The drawing under review shows one solid part. Ordinate dimensions are in mm from its lowest x, y, z. Round coordinates to 2 decimals unless told otherwise and drop trailing zeros. Order: outer loops, then holes, each group sorted by start corner. A loop starts at its lowest first (then second) coordinate and runs counter-clockwise, first axis right, second up. Notation, with made-up numbers: (84.5, 82) -> (118.5, 82) arc R29 cw to (118.5, 116) -> close; hole circle Ø5 at (33, -5). An arc over 180 degrees is marked (long way). Put each result on its own line as item: value. Start each with the question number.
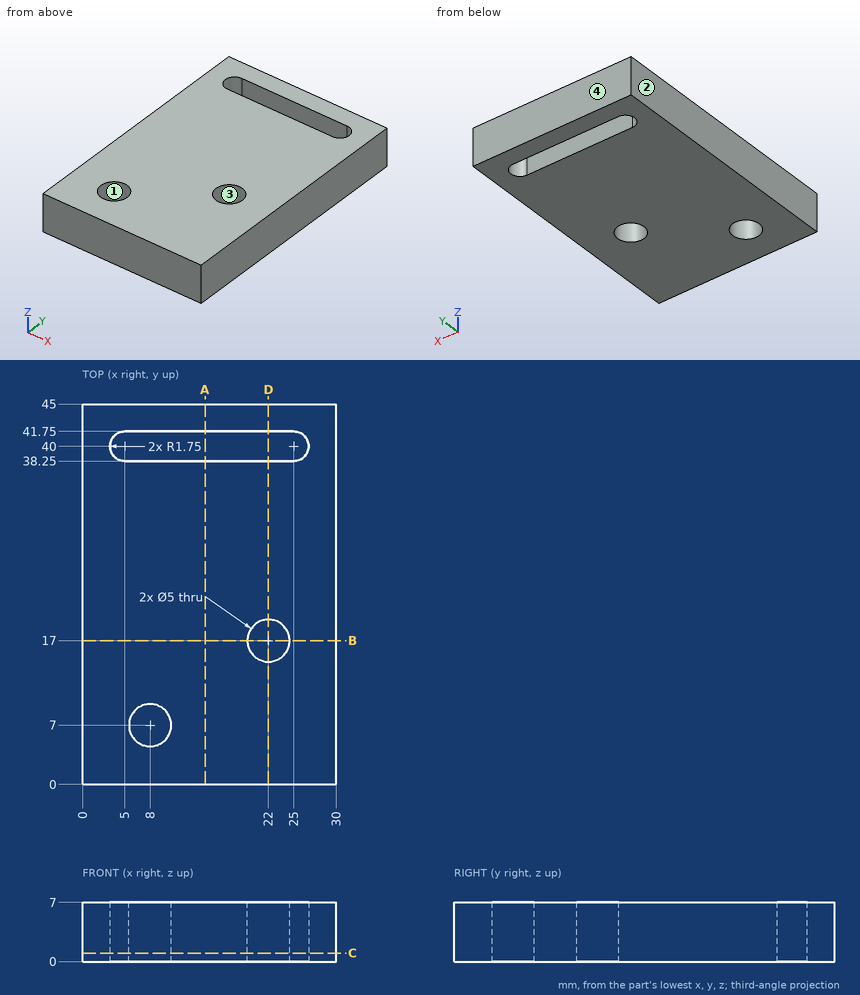
Item 1: Consider section B-B, the plane y = 17. Write out the cut boundary in (x, z), plus the area to 3 significant figures.
Item 2: Mouldability with a two-part tool opening along Y and no side actions: class the marked faces 1, 2, 3 and 4 as +Y half, -Y half, draft (parallel to the pull), parting line (faces both ways), or undercut.
Item 3: Consider section A-A, the plane x = 14.5. Write out the cut boundary in (y, z), plus the area to 4 significant figures.
Item 4: Insertion check: pin 1 Ø3 at (y, z) = (21, 5.5) entering from -X. The pin has a flat end and moves straight along its axis. Give the tip position at first contact, or say it passes through.
Item 5: For L1, parallel to Y at x = 22, z = 5.75; L2, parallel to Y at x = 8, z = 5; L3, parallel to Y at x = 11.5, z = 4, list the stretches that pass through material, from the lowest coordinate up.
Item 6: Consider section C-C, the plane z = 1. Write out the cut boundary in (x, y), plus the area to 3 significant figures.
Item 7: Consider section D-D, the plane x = 22. Write out the cut boundary in (y, z), plus the area to 4 significant figures.
Evaluation:
1. outline: (0, 0) -> (19.5, 0) -> (19.5, 7) -> (0, 7) -> close; (24.5, 0) -> (30, 0) -> (30, 7) -> (24.5, 7) -> close
1. area: 175 mm^2
2. face 1: undercut
2. face 2: draft
2. face 3: undercut
2. face 4: +Y half
3. outline: (0, 0) -> (38.25, 0) -> (38.25, 7) -> (0, 7) -> close; (41.75, 0) -> (45, 0) -> (45, 7) -> (41.75, 7) -> close
3. area: 290.5 mm^2
4. pin 1: stops at x = 0
5. L1: y = 0 to 14.5, 19.5 to 38.25, 41.75 to 45
5. L2: y = 0 to 4.5, 9.5 to 38.25, 41.75 to 45
5. L3: y = 0 to 38.25, 41.75 to 45
6. outline: (0, 0) -> (30, 0) -> (30, 45) -> (0, 45) -> close; hole (5, 38.25) -> (25, 38.25) arc R1.75 ccw to (25, 41.75) -> (5, 41.75) arc R1.75 ccw to start; hole circle Ø5 at (8, 7); hole circle Ø5 at (22, 17)
6. area: 1,230 mm^2
7. outline: (0, 0) -> (14.5, 0) -> (14.5, 7) -> (0, 7) -> close; (19.5, 0) -> (38.25, 0) -> (38.25, 7) -> (19.5, 7) -> close; (41.75, 0) -> (45, 0) -> (45, 7) -> (41.75, 7) -> close
7. area: 255.5 mm^2
